Could you check a few things on this model? Use its own coordinates, in mm. Round coordinates to 2 decimals unless told otherwise and drop trailing zeros. Loops run counter-clockwise (first coordinate to the right, second up) from the corner with the lowest first, then second, coordinate; pieces in that order, holes last.
from build123d import *

# Parameters (mm, degrees)
PLATE_OUTLINE_AND_HOLE_SKETCH_R = 10
BASE_PLATE_25MM_DEPTH           = 25
EDGE_CHAMFER_2X45DEG_SIZE       = 2


with BuildPart() as part:
    # Plate Outline and Hole Sketch → Base Plate 25mm (new body)
    with BuildSketch(Plane(origin=(0, 0, 0), x_dir=(1, 0, 0), z_dir=(0, 1, 0))):
        with BuildLine():
            Line((-140, 90), (140, 90))
            ThreePointArc((140, 90), (147.071067812, 87.071067812), (150, 80))
            Line((150, 80), (150, -80))
            ThreePointArc((150, -80), (147.071067812, -87.071067812), (140, -90))
            Line((140, -90), (-140, -90))
            ThreePointArc((-140, -90), (-147.071067812, -87.071067812), (-150, -80))
            Line((-150, -80), (-150, 80))
            ThreePointArc((-150, 80), (-147.071067812, 87.071067812), (-140, 90))
        make_face()
        with Locations(Location((-125, 65, 0), (0, 0, 270))):
            Circle(PLATE_OUTLINE_AND_HOLE_SKETCH_R, mode=Mode.SUBTRACT)
        with Locations(Location((-125, -65, 0), (0, 0, 90))):
            Circle(PLATE_OUTLINE_AND_HOLE_SKETCH_R, mode=Mode.SUBTRACT)
        with Locations(Location((125, 65, 0), (0, 0, 90))):
            Circle(PLATE_OUTLINE_AND_HOLE_SKETCH_R, mode=Mode.SUBTRACT)
        with Locations(Location((125, -65, 0), (0, 0, 270))):
            Circle(PLATE_OUTLINE_AND_HOLE_SKETCH_R, mode=Mode.SUBTRACT)
        with Locations(Location((0, 65, 0), (0, 0, 270))):
            Circle(PLATE_OUTLINE_AND_HOLE_SKETCH_R, mode=Mode.SUBTRACT)
        with Locations(Location((0, -65, 0), (0, 0, 270))):
            Circle(PLATE_OUTLINE_AND_HOLE_SKETCH_R, mode=Mode.SUBTRACT)
    extrude(amount=BASE_PLATE_25MM_DEPTH)

    # Edge Chamfer 2x45deg
    edge_chamfer_2x45deg_edges = [part.edges().sort_by_distance(p)[0] for p in [
        (-150, 0, 0),
        (-147.071067812, 0, -87.071067812),
        (0, 0, -90),
        (147.071067812, 0, -87.071067812),
        (-147.071067812, 25, -87.071067812),
        (-150, 25, 0),
        (-147.071067812, 25, 87.071067812),
        (-125, 0, -75),
        (-125, 25, -75),
        (0, 25, 90),
        (-125, 0, 75),
        (-125, 25, 75),
        (147.071067812, 25, 87.071067812),
        (125, 0, -55),
        (125, 25, -55),
        (150, 25, 0),
        (125, 0, 55),
        (125, 25, 55),
        (0, 0, -75),
        (0, 25, -75),
        (0, 0, 55),
        (0, 25, 55),
        (147.071067812, 25, -87.071067812),
        (150, 0, 0),
        (0, 25, -90),
        (147.071067812, 0, 87.071067812),
        (0, 0, 90),
        (-147.071067812, 0, 87.071067812),
    ]]
    chamfer(edge_chamfer_2x45deg_edges, length=EDGE_CHAMFER_2X45DEG_SIZE)


solid = part.part
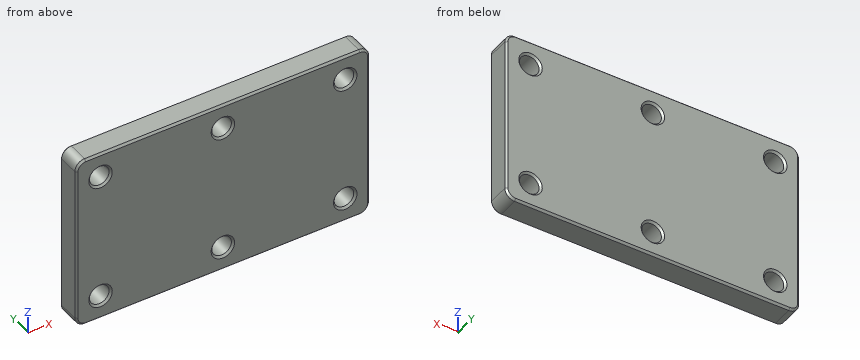
Item 1: If we section it at B-B, the plane z = -65: Count the separate pieces of the cut face and the enclosed holes in it, then the cut area to 3 significant figures.
Results list:
separate pieces: 4
enclosed holes: 0
area: 5,970 mm2
Item 2: If I drill on line 1 along Z through (x, y) = (124, 21); line 2 along X through (y, z) = (9.25, 65); line 3 along Z through (x, y) = (-120, 15), over which ranges is the centre line in solid material (lowest first)?
Results list:
line 1: z = -90 to -74.95, -55.05 to 55.05, 74.95 to 90
line 2: x = -150 to -135, -115 to -10, 10 to 115, 135 to 150
line 3: z = -90 to -73.66, -56.34 to 56.34, 73.66 to 90
Item 3: If we section it at A-A, the plane x = 125: Please give me the cut outline in (y, z).
Results list:
outline: (0, -88) - (2, -90) - (23, -90) - (25, -88) - (25, -77) - (23, -75) - (2, -75) - (0, -77) - close; (0, -53) - (2, -55) - (23, -55) - (25, -53) - (25, 53) - (23, 55) - (2, 55) - (0, 53) - close; (0, 77) - (2, 75) - (23, 75) - (25, 77) - (25, 88) - (23, 90) - (2, 90) - (0, 88) - close
Item 4: Will these pins go through, and if not, where does the flat tip stop? pin 1 (5 mm diameter, centred on x = -3.5, z = -42.5, fed in from -Y); pin 2 (16 mm diameter, centred on x = 125, z = 65, fed in from +Y).
Results list:
pin 1: stops at y = 0
pin 2: passes through
Item 5: If we section it at C-C, the plane y = 6.75: Please give me the cut outline in (x, z), then the cut area to 3 significant figures.
Results list:
outline: (-150, -80) arc R10 ccw to (-140, -90) - (140, -90) arc R10 ccw to (150, -80) - (150, 80) arc R10 ccw to (140, 90) - (-140, 90) arc R10 ccw to (-150, 80) - close; hole circle Ø20 at (-125, -65); hole circle Ø20 at (-125, 65); hole circle Ø20 at (0, -65); hole circle Ø20 at (0, 65); hole circle Ø20 at (125, -65); hole circle Ø20 at (125, 65)
area: 52,000 mm2
